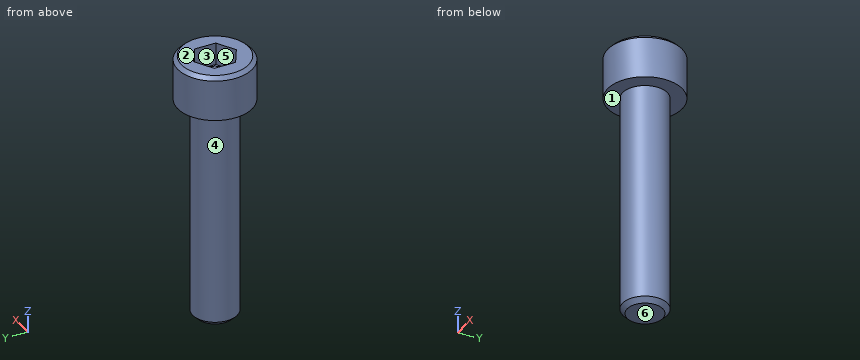
```python
from build123d import *

# Parameters (mm, degrees)
SKETCH_1_W          = 5
SKETCH_1_H          = 6
SKETCH_2_R          = 3
EXTRUDE_1_DEPTH     = 30
CUT_EXTRUDE_1_DEPTH = 3
CHAMFER_1_SIZE      = 0.5
CHAMFER_2_SIZE      = 0.6135


with BuildPart() as part:
    # 草图1 → 旋转1 (revolve)
    with BuildSketch(Plane(origin=(0, 0, 0), x_dir=(1, 0, 0), z_dir=(0, 1, 0))):
        with Locations((2.5, -3)):
            Rectangle(SKETCH_1_W, SKETCH_1_H)
    revolve(axis=Axis((0, 0, 0), (0, 0, 1)))

    # 草图2 → 凸台-拉伸1 (add)
    with BuildSketch(Plane(origin=(0, 0, 0), x_dir=(-1, 0, 0), z_dir=(0, 0, -1))):
        Circle(SKETCH_2_R)
    extrude(amount=EXTRUDE_1_DEPTH)

    # 草图3 → 切除-拉伸1 (cut)
    with BuildSketch(Plane.XY.offset(6)):
        Polygon((2.5, 1.443375673), (0, 2.886751346), (-2.5, 1.443375673), (-2.5, -1.443375673), (0, -2.886751346), (2.5, -1.443375673), align=None)
    extrude(amount=-CUT_EXTRUDE_1_DEPTH, mode=Mode.SUBTRACT)

    # 草图4 → 切除-旋转1 (revolve, cut)
    with BuildSketch(Plane.XZ):
        Polygon((2.5, 3), (0, 3), (0, 1.556624327), align=None)
    revolve(axis=Axis((0, 0, 3), (0, 0, -1)), mode=Mode.SUBTRACT)

    # 倒角1
    chamfer_1_edges = [part.edges().sort_by_distance(p)[0] for p in [
        (-5, 0, 6),
    ]]
    chamfer(chamfer_1_edges, length=CHAMFER_1_SIZE)

    # 倒角2
    chamfer_2_edges = [part.edges().sort_by_distance(p)[0] for p in [
        (3, 0, -30),
    ]]
    chamfer(chamfer_2_edges, length=CHAMFER_2_SIZE)


solid = part.part
```
Verification items for the finished model (mm, model axes). Face numbers are marked on the shaded views. A direction names the side the tool comes from. Coordinates: 2 decimals unless noted, no trailing zeros. Loops run counter-clockwise (first coordinate to the right, second up) from the corner with the lowest first, then second, coordinate; pieces in that order, holes last. Notation, with made-up numbers: (11, -36) - (23, -36) arc R14 cw to (23, -17) - close; hole circle Ø6 at (60.25, 77.25). An arc over 180 degrees is marked (long way). Return JSON: item names as keys, results as strings.
1. Tool access check on the marked faces 1, 2 and 3. Record the directions out of +Z, -Z, +X, -X, +Y, -Y that give a thin tool (end or side, any length) a straight path to the whole face; none if there is none.
Established:
{"face 1": "-Z", "face 2": "+Z, +X, -X, +Y, -Y", "face 3": "+Z"}
2. Thickness scan on L1, parallel to Y at x = 2.25, z = 4; L2, parallel to Z at x = -3.25, y = -0.75; L3, parallel to X at y = -1, z = -19. Record the ranges inside material, lowest first.
Established:
{"L1": "y = -4.47 to -1.59, 1.59 to 4.47", "L2": "z = 0 to 6", "L3": "x = -2.83 to 2.83"}
3. Mould release check, pull along X, two halves, no side actions. Record for the marked faces 4, 5 and 6: +X half, -X half, draft (parallel to the pull), parting line (faces both ways), or undercut.
Established:
{"face 4": "parting line", "face 5": "undercut", "face 6": "draft"}
4. Section check A-A, the plane z = -23.5. Record the boundary of the cut face in (x, y), then the cut area to 3 significant figures.
Established:
{"outline": "circle Ø6 at (0, 0)", "area": "28.3 mm2"}
5. Go/stop test with flat-tipped pins: pin 1 (4 mm diameter, centred on x = -3, z = -5, fed in from -Y); pin 2 (6 mm diameter, centred on x = -1.5, z = -6, fed in from +Y); pin 3 (0.6 mm diameter, centred on x = 0, y = 2.5, fed in from +Z). Record where each tip stops, or that it passes through.
Established:
{"pin 1": "stops at y = -2.83", "pin 2": "stops at y = 3", "pin 3": "stops at z = 3"}
